Source: CAD feature listing. Evaluate the final solid. Frame: model axes, mm. A direction names the side the tool comes from. Give positions to 0.01 mm unless a question says otherwise; leave off trailing zeros. Order: outer loops, then holes, each group sorted by start corner. A loop starts at its lowest first (then second) coordinate and runs counter-clockwise, first axis right, second up. Notation, with made-up numbers: M 4,86 L 17,86 A28 cw 17,117 Z; hole C -1.75,38.5 d2. An arc over 180 degrees is marked long. Answer as a JSON object with one key per item and string values. Group by question number.
1. Material intervals for L1, parallel to Z at x = -21.5, y = 54; L2, parallel to Z at x = -68, y = 0; L3, parallel to Y at x = -2.5, z = 77, sorted ascending. Write a range as [from, to].
2. Set-up query: faces 1 (the flat face through (0, 52.361, 59)), 2 (the flat face through (-41.7, 67.361, -39.4)), 3 (the flat face through (60, 60, -7.5)), 4 (the cylindrical face through (24.42, 54.42, -58.89)). Return all of +Z, -Z, +X, -X, +Y, -Y with unobstructed straight access to the full face (end or side cutting, diameter ignored); none if empty.
3. Section query B-B (y = 47). Output: boundary loops of the cut face in (x, z), plus the area to 3 significant figures.
4. Pin query (flat end, axial travel): P1, Ø2, axis at y = 51.5, z = -19.5, coming from the -X side; P2, Ø4.5, axis at y = 60.5, z = 60, coming from the -X side; P3, Ø4, axis at y = 19.5, z = 29, coming from the -X side; P4, Ø24, axis at x = 0, z = 86.25, coming from the -Y side. Return the tip coordinate at first contact, or that it passes through.
5. Section query C-C (x = -71.5). Count the separate pieces of the cut face and the enclosed holes in it, plus the area to 3 significant figures.
6. Pull-direction query (Y, two-part tool) for faces 5 (the cylindrical face through (-2.8, 9.26, 63.69)), 6 (the flat face through (50, 11.111, -40)), 7 (the flat face through (0, 52.361, -59)), 8 (the cylindrical face through (68.454, -0.958, -38.943)); classes: +Y half, -Y half, draft (parallel to the pull), parting line (faces both ways), or undercut.
7. Section query A-A (z = 0). Output: boundary loops of the cut face in (x, y) (3 decimals).
from build123d import *

# Parameters (mm, degrees)
SKETCH2_W          = 20
SKETCH2_H          = 8
SKETCH2_W_2        = 8
SKETCH2_H_2        = 20
CUT_EXTRUDE1_DEPTH = 8
SKETCH3_R          = 4
CUT_EXTRUDE2_DEPTH = 100
SCALE_1_SCALE      = 1.875


with BuildPart() as part:
    # Sketch1 → Revolve1 (revolve)
    with BuildSketch(Plane.XY, mode=Mode.PRIVATE) as revolve1_sk:
        with BuildLine():
            Line((32, 0), (54, 0))
            Line((54, 0), (56, 2))
            Line((56, 2), (56, 9))
            Line((56, 9), (36, 9))
            Line((36, 9), (34, 9))
            Line((34, 9), (34, 11))
            Line((34, 11), (36, 11))
            Line((36, 11), (36, 27))
            Line((36, 27), (34, 27))
            Line((34, 27), (34, 41))
            Line((34, 41), (30.5, 41))
            Line((30.5, 41), (26.45024814, 15.502481405))
            ThreePointArc((26.45024814, 15.502481405), (24.830088793, 12.292737332), (21.475062189, 11))
            Line((21.475062189, 11), (0, 11))
            Line((0, 11), (0, 2))
            Line((0, 2), (31, 2))
            Line((31, 2), (32, 0))
        make_face()
    revolve(revolve1_sk.sketch.rotate(Axis((0, 2, 0), (0, 1, 0)), 90), axis=Axis((0, 2, 0), (0, 1, 0)))

    # Sketch2 → Cut-Extrude1 (cut)
    with BuildSketch(Plane(origin=(0, 41, 0), x_dir=(1, 0, 0), z_dir=(0, 1, 0))):
        with Locations((27.262332301, 0)):
            Rectangle(SKETCH2_W, SKETCH2_H)
        with Locations((0, 27.262332301)):
            Rectangle(SKETCH2_W_2, SKETCH2_H_2)
        with Locations((0, -27.262332301)):
            Rectangle(SKETCH2_W_2, SKETCH2_H_2)
        with Locations((-27.262332301, 0)):
            Rectangle(SKETCH2_W, SKETCH2_H)
    extrude(amount=-CUT_EXTRUDE1_DEPTH, mode=Mode.SUBTRACT)

    # Sketch3 → Cut-Extrude2 (cut)
    with BuildSketch(Plane(origin=(0, 41, 0), x_dir=(1, 0, 0), z_dir=(0, 1, 0))):
        with Locations(Location((0, 46, 0), (0, 0, 270))):
            Circle(SKETCH3_R)
        with Locations(Location((40.056631801, 22.615619575, 0), (0, 0, 270))):
            Circle(SKETCH3_R)
        with Locations(Location((-39.837168574, 23, 0), (0, 0, 270))):
            Circle(SKETCH3_R)
        with Locations(Location((-39.837168574, -23, 0), (0, 0, 270))):
            Circle(SKETCH3_R)
        with Locations(Location((0, -46, 0), (0, 0, 270))):
            Circle(SKETCH3_R)
        with Locations(Location((40.056631801, -22.615619575, 0), (0, 0, 270))):
            Circle(SKETCH3_R)
    extrude(amount=-CUT_EXTRUDE2_DEPTH, mode=Mode.SUBTRACT)


with BuildPart() as part_1:
    # Scale 1: scaled about (-0.001562363, 10.8729077, 0)
    add(part.part.scale(SCALE_1_SCALE).moved(Location((0.001367068, -9.513794238, 0))))


solid = part_1.part
Answer sheet:
{
 "1": {"L1": "[-60.01, -50.69], [50.69, 60.01]", "L2": "[-80.01, -46.51], [-39.74, 39.74], [46.51, 80.01]", "L3": "[-9.51, 7.36]"},
 "2": {"face 1": "+Z, -Z, +Y", "face 2": "+Z, -Z, +X, -X, +Y", "face 3": "+X, -X, +Y", "face 4": "+Y"},
 "3": {"outline": "C 0,0 d127.5; hole C 0,0 d107.91", "area": "3,620 mm^2"},
 "4": {"P1": "x = -61.01", "P2": "x = -27", "P3": "x = -61.86", "P4": "y = -9.51"},
 "5": {"separate pieces": "3", "enclosed holes": "0", "area": "2,120 mm^2"},
 "6": {"face 5": "undercut", "face 6": "undercut", "face 7": "+Y half", "face 8": "draft"},
 "7": {"outline": "M -104.999,-5.764 L -101.249,-9.514 L -59.999,-9.514 L -58.124,-5.764 L 58.126,-5.764 L 60.001,-9.514 L 101.251,-9.514 L 105.001,-5.764 L 105.001,7.361 L 63.751,7.361 L 63.751,11.111 L 67.501,11.111 L 67.501,41.111 L 63.751,41.111 L 63.751,52.361 L 54.806,52.361 L 49.596,19.553 A9.375 cw 40.267,11.111 L -40.264,11.111 A9.375 cw -49.593,19.553 L -54.804,52.361 L -63.749,52.361 L -63.749,41.111 L -67.499,41.111 L -67.499,11.111 L -63.749,11.111 L -63.749,7.361 L -104.999,7.361 Z"}
}
